Source: CAD feature listing. Evaluate the final solid. Frame: model axes, mm. Coordinates: 2 decimals unless noted, no trailing zeros. Order: outer loops, then holes, each group sorted by start corner. A loop starts at its lowest first (then second) coordinate and runs counter-clockwise, first axis right, second up. Notation, with made-up numbers: (16, 76) -> (47, 76) arc R17 ccw to (47, 100) -> close; hole circle Ø10 at (-23, -28). An arc over 180 degrees is marked (long way). Write item = value, one per line. Start each with the question number.
Item 1: Mould query, pull axis Z, two halves, no side actions, for faces 1 (the flat face through (0, 7, -40)), 2 (the cylindrical face through (-0.74, 7.6, 3.32)), 3 (the flat face through (-40, 7, 0)). Classes: released by +Z, released by -Z, zero draft, split by the parting line, or undercut.
Item 2: Section query B-B (x = 0). Output: boundary loops of the cut face in (y, z), then the cut area to 3 significant figures.
Item 3: Ray query, line 1 along Z through (x, y) = (0, 8.25); line 2 along Z through (x, y) = (-3, 10.5); line 3 along X through (y, z) = (0.75, 2). Return the intervals inside material, ascending. Write a range as [from, to].
Item 4: Contact query for a flat-ended pin moving along its axis: pin 1 (11 mm diameter, centred on x = 0, z = 0, fed in from -Y). Output: stop coordinate, or through.
Item 5: Section query A-A (z = 0). Output: boundary loops of the cut face in (x, y), then the cut area to 3 significant figures.
```python
from build123d import *

# Parameters (mm, degrees)
SKETCH_1_W             = 80
SKETCH_1_H             = 80
EXTRUDE_1_DEPTH        = 15
FILLET_1_R             = 5
HOLE_WIZARD_M8_1_D     = 6.8
HOLE_WIZARD_M8_1_DEPTH = 19.75
HOLE_WIZARD_M8_1_TIP   = 2.042926105


with BuildPart() as part:
    # 草图1 → 凸台-拉伸1 (new body)
    with BuildSketch(Plane(origin=(0, 0, 0), x_dir=(1, 0, 0), z_dir=(0, 1, 0))):
        Rectangle(SKETCH_1_W, SKETCH_1_H)
    extrude(amount=EXTRUDE_1_DEPTH)

    # 圆角1
    fillet_1_edges = [part.edges().sort_by_distance(p)[0] for p in [
        (40, 7.5, 40),
        (-40, 7.5, 40),
        (-40, 7.5, -40),
        (40, 7.5, -40),
    ]]
    fillet(fillet_1_edges, radius=FILLET_1_R)

    # M8 螺纹孔1
    with Locations(Plane(origin=(0, 0, 0), x_dir=(-1, 0, 0), z_dir=(0, -1, 0))):
        with Locations((0, 0)):
            Hole(HOLE_WIZARD_M8_1_D / 2, depth=HOLE_WIZARD_M8_1_DEPTH)
            with Locations((0, 0, -(HOLE_WIZARD_M8_1_DEPTH + HOLE_WIZARD_M8_1_TIP / 2))):  # 118° drill point
                Cone(0, HOLE_WIZARD_M8_1_D / 2, HOLE_WIZARD_M8_1_TIP, mode=Mode.SUBTRACT)


solid = part.part
```
Computed:
q1.face_1 = released by -Z
q1.face_2 = undercut
q1.face_3 = zero draft
q2.outline = (0, -40) -> (15, -40) -> (15, -3.4) -> (0, -3.4) -> close; (0, 3.4) -> (15, 3.4) -> (15, 40) -> (0, 40) -> close
q2.area = 1,100 mm^2
q3.line_1 = [-40, -3.4], [3.4, 40]
q3.line_2 = [-40, -1.6], [1.6, 40]
q3.line_3 = [-40, -2.75], [2.75, 40]
q4.pin_1 = 0
q5.outline = (-40, 0) -> (-3.4, 0) -> (-3.4, 15) -> (-40, 15) -> close; (3.4, 0) -> (40, 0) -> (40, 15) -> (3.4, 15) -> close
q5.area = 1,100 mm^2
